```python
from build123d import *

# Parameters (mm, degrees)
CHAMFER1_SIZE = 0.5


with BuildPart() as part:
    # Sketch1 → Revolve1 (revolve)
    with BuildSketch(Plane.XY):
        Polygon((-139.286891893, -435.685707644), (-139.686891893, -435.685707644), (-139.686891893, -417.685707644), (-145.536891893, -417.685707644), (-145.536891893, -412.685707644), (-133.036891893, -412.685707644), (-133.036891893, -447.685707644), (-139.286891893, -447.685707644), align=None)
    revolve(axis=Axis((-133.036891893, -412.685707644, 0), (0, -1, 0)))

    # Chamfer1
    chamfer1_edges = [part.edges().sort_by_distance(p)[0] for p in [
        (-120.536891893, -412.685707644, 0),
        (-120.536891893, -417.685707644, 0),
        (-126.786891893, -447.685707644, 0),
    ]]
    chamfer(chamfer1_edges, length=CHAMFER1_SIZE)


solid = part.part
```
CAD build for the part. Positions are in the model's coordinates, mm. A direction names the side the tool comes from. Coordinates: 2 decimals unless noted, no trailing zeros. Order: outer loops, then holes, each group sorted by start corner. A loop starts at its lowest first (then second) coordinate and runs counter-clockwise, first axis right, second up.
(1) Saw through at B-B, the plane y = -444. Write the cut outline in (x, z), and give its area (3 significant figures).
Solution:
outline: circle Ø12.5 at (-133.04, 0)
area: 123 mm2
(2) Saw through at A-A, the plane z = 0. Write the cut outline in (x, y).
Solution:
outline: (-145.54, -417.19) - (-145.04, -417.69) - (-139.69, -417.69) - (-139.69, -435.69) - (-139.29, -435.69) - (-139.29, -447.19) - (-138.79, -447.69) - (-127.29, -447.69) - (-126.79, -447.19) - (-126.79, -435.69) - (-126.39, -435.69) - (-126.39, -417.69) - (-121.04, -417.69) - (-120.54, -417.19) - (-120.54, -413.19) - (-121.04, -412.69) - (-145.04, -412.69) - (-145.54, -413.19) - close
(3) Pin check, flat tips, straight feed: pin 1 Ø3 at (x, y) = (-132, -424) entering from +Z; pin 2 Ø4 at (y, z) = (-420, 4) entering from +X; pin 3 Ø8 at (y, z) = (-426, 7.5) entering from -X. Stop position of each tip, or through.
Solution:
pin 1: stops at z = 6.65
pin 2: stops at x = -126.69
pin 3: stops at x = -138.69
(4) Which spindle directions (+Z, -Z, +X, -X, +Y, -Y) get a long thin tool onto all of the face, cutting with end or side? Do faces 1 (the face through (-133, -412.686, 0)), 2 (the face through (-139.38, -426.56, -2)). Say none if no direction does.
Solution:
face 1: +Z, -Z, +X, -X, +Y
face 2: -Y
(5) Drill centre lines: L1, parallel to Y at x = -125, z = 8.5; L2, parallel to Z at x = -129.5, y = -429; L3, parallel to X at y = -440, z = -3.5. Where is each one in solid material? Low to high.
Solution:
L1: y = -417.69 to -412.69
L2: z = -5.63 to 5.63
L3: x = -138.21 to -127.86
